Could you check a few things on this model? Use its own coordinates, in mm. A direction names the side the tool comes from. Give positions to 0.01 mm unless a question says otherwise; leave off trailing zeros. Order: outer loops, then holes, each group sorted by start corner. A loop starts at its lowest first (then second) coordinate and runs counter-clockwise, first axis right, second up. Notation, with made-up numbers: (50, -17.5) -> (75, -17.5) arc R16 cw to (75, 9.5) -> close; hole circle Ø1 at (-17, -34.75). An arc over 180 degrees is marked (long way). One line per item, written item: value.
```python
from build123d import *

# Parameters (mm, degrees)
SKETCH1_R               = 4
BOSS_EXTRU_1_DEPTH      = 3
SKETCH2_R               = 4
BOSS_EXTRU_2_DEPTH      = 3
CUT_EXTRUDE1_DEPTH      = 10
CUT_EXTRUDE1_DEPTH_BACK = 100.231025361
SKETCH3_R               = 20.05
BOSS_EXTRU_3_REACH      = 101.231
SKETCH5_R               = 23.05
SKETCH5_R_2             = 20.05


with BuildPart() as part:
    # Sketch1 → Boss.-Extru.1 (new body)
    with BuildSketch(Plane.XY):
        with BuildLine():
            Line((-83.689862838, 93.775756105), (-30.050252532, 40.136145798))
            ThreePointArc((-30.050252532, 40.136145798), (-25.832748997, 37.318100031), (-20.857864376, 36.328533954))
            Line((-20.857864376, 36.328533954), (20.857864376, 36.328533954))
            ThreePointArc((20.857864376, 36.328533954), (25.832748997, 37.318100031), (30.050252532, 40.136145798))
            Line((30.050252532, 40.136145798), (83.689862838, 93.775756105))
            ThreePointArc((83.689862838, 93.775756105), (85.154328933, 97.311290011), (83.689862838, 100.846823917))
            Line((83.689862838, 100.846823917), (78.033008589, 106.503678166))
            ThreePointArc((78.033008589, 106.503678166), (74.497474683, 107.96814426), (70.961940777, 106.503678166))
            Line((70.961940777, 106.503678166), (25.807611845, 61.349349234))
            ThreePointArc((25.807611845, 61.349349234), (23.536648403, 59.831939975), (20.857864376, 59.299096702))
            Line((20.857864376, 59.299096702), (-20.857864376, 59.299096702))
            ThreePointArc((-20.857864376, 59.299096702), (-23.536648403, 59.831939975), (-25.807611845, 61.349349234))
            Line((-25.807611845, 61.349349234), (-70.961940777, 106.503678166))
            ThreePointArc((-70.961940777, 106.503678166), (-74.497474683, 107.96814426), (-78.033008589, 106.503678166))
            Line((-78.033008589, 106.503678166), (-83.689862838, 100.846823917))
            ThreePointArc((-83.689862838, 100.846823917), (-85.154328933, 97.311290011), (-83.689862838, 93.775756105))
        make_face()
        with Locations((-73.083261121, 95.897076449)):
            Circle(SKETCH1_R, mode=Mode.SUBTRACT)
        with Locations(Location((73.083261121, 95.897076449, 0), (0, 0, 180))):
            Circle(SKETCH1_R, mode=Mode.SUBTRACT)
    extrude(amount=BOSS_EXTRU_1_DEPTH)


with BuildPart() as body_2:
    # Sketch2 → Boss.-Extru.2 (new body)
    with BuildSketch(Plane(origin=(0, 0, -12), x_dir=(-1, 0, 0), z_dir=(0, 0, -1))):
        with BuildLine():
            Line((-25.814562691, 61.342398387), (-70.968891623, 106.49672732))
            ThreePointArc((-70.968891623, 106.49672732), (-74.504425529, 107.961193414), (-78.039959435, 106.49672732))
            Line((-78.039959435, 106.49672732), (-83.696813685, 100.839873071))
            ThreePointArc((-83.696813685, 100.839873071), (-85.161279779, 97.304339165), (-83.696813685, 93.768805259))
            Line((-83.696813685, 93.768805259), (-30.057203378, 40.129194952))
            ThreePointArc((-30.057203378, 40.129194952), (-25.839699843, 37.311149185), (-20.864815223, 36.321583107))
            Line((-20.864815223, 36.321583107), (20.85091353, 36.321583107))
            ThreePointArc((20.85091353, 36.321583107), (25.825798151, 37.311149185), (30.043301685, 40.129194952))
            Line((30.043301685, 40.129194952), (83.682911992, 93.768805259))
            ThreePointArc((83.682911992, 93.768805259), (85.147378086, 97.304339165), (83.682911992, 100.839873071))
            Line((83.682911992, 100.839873071), (78.026057743, 106.49672732))
            ThreePointArc((78.026057743, 106.49672732), (74.490523837, 107.961193414), (70.954989931, 106.49672732))
            Line((70.954989931, 106.49672732), (25.800660998, 61.342398387))
            ThreePointArc((25.800660998, 61.342398387), (23.529697556, 59.824989128), (20.85091353, 59.292145856))
            Line((20.85091353, 59.292145856), (-20.864815223, 59.292145856))
            ThreePointArc((-20.864815223, 59.292145856), (-23.543599249, 59.824989128), (-25.814562691, 61.342398387))
        make_face()
        with Locations((-73.090211967, 95.890125602)):
            Circle(SKETCH2_R, mode=Mode.SUBTRACT)
        with Locations(Location((73.076310274, 95.890125602, 0), (0, 0, 180))):
            Circle(SKETCH2_R, mode=Mode.SUBTRACT)
    extrude(amount=BOSS_EXTRU_2_DEPTH)


with BuildPart() as cut_extrude1_tool:
    # Sketch3 → Cut-Extrude1 (new, two sides: drawn at the far end of the back side and taken through both)
    with BuildSketch(Plane(origin=(0, 59.292145856, 0), x_dir=(1, 0, 0), z_dir=(0, 1, 0)).offset(-CUT_EXTRUDE1_DEPTH_BACK)):
        with Locations((-0.00205312, 6.000001678)):
            Circle(SKETCH3_R)
    extrude(amount=CUT_EXTRUDE1_DEPTH + CUT_EXTRUDE1_DEPTH_BACK)


with BuildPart() as part_1:
    add(part.part)

    # Cut-Extrude1: cut by cut_extrude1_tool
    add(cut_extrude1_tool.part, mode=Mode.SUBTRACT)


with BuildPart() as body_2_1:
    add(body_2.part)

    # Cut-Extrude1: cut by cut_extrude1_tool
    add(cut_extrude1_tool.part, mode=Mode.SUBTRACT)


with BuildPart() as cut_extrude1_piece_1:
    # of the separate pieces the step leaves, piece 1, a body of its own (cut_extrude1_pieces)
    add(part_1.part.solids().sort_by_distance((19.129138162, 36.328533954, 0))[0])


with BuildPart() as cut_extrude1_piece_2:
    # of the separate pieces the step leaves, piece 2, a body of its own (cut_extrude1_pieces)
    add(part_1.part.solids().sort_by_distance((-83.689862838, 93.775756105, 0))[0])


with BuildPart() as cut_extrude1_piece_1_of_body_2:
    # of the separate pieces the step leaves, piece 1, a body of its own (cut_extrude1_pieces_of_body_2)
    add(body_2_1.part.solids().sort_by_distance((25.814562691, 61.342398387, -12))[0])


with BuildPart() as cut_extrude1_piece_2_of_body_2:
    # of the separate pieces the step leaves, piece 2, a body of its own (cut_extrude1_pieces_of_body_2)
    add(body_2_1.part.solids().sort_by_distance((-20.85091353, 59.292145856, -12))[0])

    # Boss.-Extru.3: up to this face of the body (flat: up to its plane)
    boss_extru_3_end = Plane(cut_extrude1_piece_2_of_body_2.part.faces().sort_by_distance((-19.684947548, 36.321583107, -13.633103381))[0])
    # Sketch5 → Boss.-Extru.3 (add, up to the picked face)
    with BuildSketch(Plane(origin=(0, 59.292145856, 0), x_dir=(1, 0, 0), z_dir=(0, 1, 0)), mode=Mode.PRIVATE) as boss_extru_3_sk1:
        with Locations(Location((-0.00205312, 6.000001678, 0), (0, 0, 180))):
            Circle(SKETCH5_R)
        with Locations(Location((-0.00205312, 6.000001678, 0), (0, 0, 342.587320704))):
            Circle(SKETCH5_R_2, mode=Mode.SUBTRACT)
    boss_extru_3_tool1 = split(extrude(boss_extru_3_sk1.sketch, amount=-BOSS_EXTRU_3_REACH, mode=Mode.PRIVATE), bisect_by=boss_extru_3_end, keep=Keep.BOTH, mode=Mode.PRIVATE)

    add(cut_extrude1_piece_1.part)  # Boss.-Extru.3 merges Cut-Extrude1 piece 1

    add(cut_extrude1_piece_2.part)  # Boss.-Extru.3 merges Cut-Extrude1 piece 2

    add(cut_extrude1_piece_1_of_body_2.part)  # Boss.-Extru.3 merges Cut-Extrude1 piece 1 of body 2
    add(boss_extru_3_tool1.solids().sort_by(Axis((22.395994, 59.292146, -6.000002), (0, -1, 0)))[0])


solid = cut_extrude1_piece_2_of_body_2.part
```
1) Suppose I cut it at A-A, the plane z = -3. Write out the boundary of the cut face in (x, y), then the cut area to 3 significant figures.
Answer below:
outline: (-22.86, 36.32) -> (-19.83, 36.32) -> (-19.83, 59.29) -> (-22.86, 59.29) -> close; (19.82, 36.32) -> (22.85, 36.32) -> (22.85, 59.29) -> (19.82, 59.29) -> close
area: 139 mm2
2) For faces 1 (the cylindrical face through (-25.934, 37.356, -13.479)), 2 (the cylindrical face through (-85.147, 97.249, -13.479)), 3 (the flat face through (20, 59.299, 1)), which set-ups out of +Z, -Z, +X, -X, +Y, -Y let a thin tool reach every point of the face, with its end or its side?
Answer below:
face 1: -Z, -X, -Y
face 2: +Z, -Z, -X
face 3: +Z, -Z, +Y
3) For P1, Ø12, axis at y = 93.5, z = -7, coming from the +X side; P2, Ø9, axis at x = 73.08, y = 95.9, coming from the -Z side; P3, Ø8.5, axis at x = 4.5, z = -21.5, coming from the +Y side, each with a flat end and sliding along its axis, tell me the tip position at first contact or that it passes through.
Answer below:
P1: stops at x = 85.14
P2: stops at z = -15
P3: stops at y = 59.29
4) We'd pull the mould along Z, two halves only. Please class faces 4 (the flat face through (-50, 72, 0)), 5 (the flat face through (-50, 72, -15)), 6 (the flat face through (48.7, 84.24, 1.48)): +Z half, -Z half, draft (parallel to the pull), parting line (faces both ways), or undercut.
Answer below:
face 4: undercut
face 5: -Z half
face 6: draft
5) Suppose I cut it at B-B, the plane x = 7. Write out the boundary of the cut face in (y, z).
Answer below:
outline: (36.32, -27.96) -> (59.29, -27.96) -> (59.29, -24.79) -> (36.32, -24.79) -> close; (36.32, 12.79) -> (59.29, 12.79) -> (59.29, 15.96) -> (36.32, 15.96) -> close
6) If I drill on line 1 along X through (y, z) = (44.5, -7); line 2 along Z through (x, y) = (-31, 64); line 3 along X through (y, z) = (88.5, 1.5), over which ranges is the centre line in solid material (lowest first)?
Answer below:
line 1: x = -23.03 to -20.03, 20.02 to 23.03
line 2: z = -15 to -12, 0 to 3
line 3: x = -78.41 to -52.96, 52.96 to 78.41
7) Suppose I cut it at C-C, the plane y = 44. Write out the boundary of the cut face in (x, z), then the cut area to 3 significant figures.
Answer below:
outline: (-33.91, -15) -> (-21.22, -15) arc R23.05 ccw to (21.22, -15) -> (33.93, -15) -> (33.93, -12) -> (22.25, -12) arc R23.05 ccw to (22.25, 0) -> (33.91, 0) -> (33.91, 3) -> (21.22, 3) arc R23.05 ccw to (-21.22, 3) -> (-33.91, 3) -> (-33.91, 0) -> (-22.26, 0) arc R23.05 ccw to (-22.26, -12) -> (-33.91, -12) -> close; hole circle Ø40.1 at (0, -6)
area: 552 mm2
8) Suppose I cut it at D-D, the plane x = 73.5. Write out the boundary of the cut face in (y, z), then the cut area to 3 significant figures.
Answer below:
outline: (83.57, -15) -> (91.91, -15) -> (91.91, -12) -> (83.57, -12) -> close; (83.59, 0) -> (91.92, 0) -> (91.92, 3) -> (83.59, 3) -> close; (99.87, -15) -> (107.86, -15) -> (107.86, -12) -> (99.87, -12) -> close; (99.88, 0) -> (107.87, 0) -> (107.87, 3) -> (99.88, 3) -> close
area: 98.0 mm2
